```python
from build123d import *

# Parameters (mm, degrees)
SKETCH_1_R          = 425
SKETCH_1_R_2        = 355
EXTRUDE_2_DEPTH     = 12
SKETCH_3_R          = 385
SKETCH_3_R_2        = 370
EXTRUDE_3_DEPTH     = 36
SWEEP_2_PROFILE_R   = 8
SKETCH_23_W         = 4.5
SKETCH_23_H         = 385
SKETCH_24_R         = 9
CUT_EXTRUDE_1_DEPTH = 15


with BuildPart() as part:
    # 草图1 → 凸台-拉伸2 (new body)
    with BuildSketch(Plane.XY):
        Circle(SKETCH_1_R)
        Circle(SKETCH_1_R_2, mode=Mode.SUBTRACT)
    extrude(amount=EXTRUDE_2_DEPTH)

    # 草图3 → 凸台-拉伸3 (add)
    with BuildSketch(Plane(origin=(0, 0, 0), x_dir=(-1, 0, 0), z_dir=(0, 0, -1))):
        with Locations(Location((0, 0, 0), (0, 0, 180))):
            Circle(SKETCH_3_R)
        Circle(SKETCH_3_R_2, mode=Mode.SUBTRACT)
    extrude(amount=EXTRUDE_3_DEPTH)

    # 切除-扫描2: sweep along a path in 草图4
    with BuildLine(Plane.XY.offset(-18)) as sweep_2_path:
        CenterArc((0, 0), 370, 0, 360)
    # 切除-扫描2 profile (on start of the path) → 切除-扫描2 (sweep, cut)
    with BuildSketch(Plane(origin=(370, 0, -18), x_dir=(0, 0, 1), z_dir=(0, 1, 0))):
        Circle(SWEEP_2_PROFILE_R)
    sweep(path=sweep_2_path.line, mode=Mode.SUBTRACT)

    # 草图23 → M10x1.0 螺纹孔1 (revolve, cut)
    with BuildSketch(Plane(origin=(0, 0, -18), x_dir=(0, 0, 1), z_dir=(0, 1, 0))):
        with Locations((2.25, 192.5)):
            Rectangle(SKETCH_23_W, SKETCH_23_H)
    revolve(axis=Axis((-6.35, 0, -18), (1, 0, 0)), mode=Mode.SUBTRACT)

    # 草图24 → 切除-拉伸1 (cut)
    with BuildSketch(Plane(origin=(0, 0, 0), x_dir=(-1, 0, 0), z_dir=(0, 0, -1))):
        with Locations((-125, -389.430353208)):
            Circle(SKETCH_24_R)
        with Locations((125, -389.430353208)):
            Circle(SKETCH_24_R)
        with Locations((-255.40902876, -319.448318243)):
            Circle(SKETCH_24_R)
        with Locations((255.40902876, -319.448318243)):
            Circle(SKETCH_24_R)
        with Locations((-125, 389.430353208)):
            Circle(SKETCH_24_R)
        with Locations((125, 389.430353208)):
            Circle(SKETCH_24_R)
        with Locations((342.768366919, 223.138626507)):
            Circle(SKETCH_24_R)
        with Locations((-342.768366919, 223.138626507)):
            Circle(SKETCH_24_R)
    extrude(amount=-CUT_EXTRUDE_1_DEPTH, mode=Mode.SUBTRACT)


solid = part.part
```
Here's how the part is built. I have some questions about the finished solid (model axes, mm). A direction names the side the tool comes from. Give positions to 0.01 mm unless a question says otherwise; leave off trailing zeros. Loops run counter-clockwise (first coordinate to the right, second up) from the corner with the lowest first, then second, coordinate; pieces in that order, holes last. Notation, with made-up numbers: M -36,70 L 3,70 A9 cw 3,87 Z; hole C 73.5,11.5 d6. An arc over 180 degrees is marked long. Return JSON: item names as keys, results as strings.
Item 1: Please list where these lines run through material, in increasing order: line 1 (X direction, y = 0, z = -2.75); line 2 (Y direction, x = 125, z = 4.25); line 3 (Y direction, x = 12, z = -6).
A:
{"line 1": "x = -385 to -370, 370 to 385", "line 2": "y = -406.2 to -398.43, -380.43 to -332.26, 332.26 to 380.43, 398.43 to 406.2", "line 3": "y = -384.81 to -369.81, 369.81 to 384.81"}
Item 2: I'm going to push flat-ended pins straight in: pin 1 Ø1 at (y, z) = (143, -11.5) entering from +X; pin 2 Ø5 at (x, z) = (165, 7) entering from +Y; pin 3 Ø20.5 at (x, y) = (125, -389.43) entering from -Z. Where does each tip first touch, or does it pass through?
A:
{"pin 1": "stops at x = 357.66", "pin 2": "stops at y = 392.71", "pin 3": "stops at z = 0"}
Item 3: Imagine slicing it at A-A on x = 0. List the corners of the cut face in (y, z) for me.
A:
{"outline": "M -425,0 L -385,0 L -385,-36 L -370,-36 L -370,-26 A8 cw -370,-10 L -370,0 L -355,0 L -355,12 L -425,12 Z; M 355,0 L 370,0 L 370,-10 A8 cw 370,-26 L 370,-36 L 385,-36 L 385,0 L 425,0 L 425,12 L 355,12 Z"}
Item 4: On a 3-axis mill with a long thin cutter (end or side, diameter ignored), from which of +Z, -Z, +X, -X, +Y, -Y can I reach the whole of each face in a straight line? I mean faces 4 (the flat face through (-201, -316, -36)), 5 (the flat face through (-139, 331, 0)). Say none if no direction works.
A:
{"face 4": "-Z, +X, -X, +Y, -Y", "face 5": "-Z"}
Item 5: Thinking about a two-plate mould opening in Y: for faces 1 (the cylindrical face through (-55.327, 421.383, 5.916)), 2 (the cylindrical face through (-281.716, -216.012, 5.916)), 3 (the flat face through (92, 348, 12)), which applies, released by +Y, released by -Y, zero draft, split by the parting line, or undercut?
A:
{"face 1": "split by the parting line", "face 2": "undercut", "face 3": "zero draft"}
